For this review, take the finished solid that the model builds, in its own axes (mm). Face numbers are marked on the shaded views. Round coordinates to 2 decimals unless told otherwise and drop trailing zeros. Order: outer loops, then holes, each group sorted by start corner. A loop starts at its lowest first (then second) coordinate and runs counter-clockwise, first axis right, second up. Notation, with made-up numbers: (-10.75, -20) -> (32.25, -20) arc R22 cw to (32.25, 15) -> close; hole circle Ø4 at (6, 67.5). An arc over 180 degrees is marked (long way). Use a Markdown table: item, result. Add a question column.
1) Clearance check with flat-ended pins moving along their axes: P1, Ø2, axis at x = -232, z = -14.5, coming from the +Y side; P2, Ø1, axis at x = -254, z = -40, coming from the -Y side; P3, Ø12, axis at x = -193.5, y = 17, coming from the +Z side (3 decimals). State where each tip first meets the part, or that it passes through.
2) Wall thickness on line 1 along X through (y, z) = (-27, 65); line 2 along Y through (x, z) = (-233.5, 6.5); line 3 along Z through (x, y) = (-229.5, 36): over which ranges is each line inside the solid? List them lowest first. Write a range as [from, to].
3) Consider section D-D (x = -282.5). State the section outline as (y, z) points, plus the area to 3 significant figures.
4) Draft analysis for pull direction X (two halves, no side actions). For the marked faces 1, 2 and 3, state which applies: pulls with the +X half, pulls with the -X half, needs draft (parallel to the pull), parting line crosses it, or undercut.
5) Consider section A-A (z = 59.5). State the section outline as (x, y) points.
6) Consider section B-B (y = 0). State the section outline as (x, z) points.
7) Consider section C-C (z = 25). State the section outline as (x, y) points, plus the area to 3 significant figures.
```python
from build123d import *

# Parameters (mm, degrees)
SKETCH_1_4_R        = 75
BOSS_EXTRUDE1_DEPTH = 18
SKETCH_1_3_R        = 50
BOSS_EXTRUDE2_DEPTH = 311
BOSS_EXTRUDE3_START = -329
SKETCH_1_4_2_R      = 75
BOSS_EXTRUDE3_DEPTH = 18


with BuildPart() as part:
    # Sketch 1_4 → Boss-Extrude1 (new body)
    with BuildSketch(Plane(origin=(0, 0, 0), x_dir=(0, 0, -1), z_dir=(1, 0, 0))):
        Circle(SKETCH_1_4_R)
    extrude(amount=BOSS_EXTRUDE1_DEPTH)

    # 草图1<3> → Boss-Extrude2 (add)
    with BuildSketch(Plane(origin=(0, 0, 0), x_dir=(0, 0, -1), z_dir=(1, 0, 0))):
        Circle(SKETCH_1_3_R)
    extrude(amount=-BOSS_EXTRUDE2_DEPTH)

    # Sketch 1_4 2 → Boss-Extrude3 (add)
    with BuildSketch(Plane(origin=(0, 0, 0), x_dir=(0, 0, -1), z_dir=(1, 0, 0)).offset(BOSS_EXTRUDE3_START)):
        Circle(SKETCH_1_4_2_R)
    extrude(amount=BOSS_EXTRUDE3_DEPTH)


solid = part.part
```
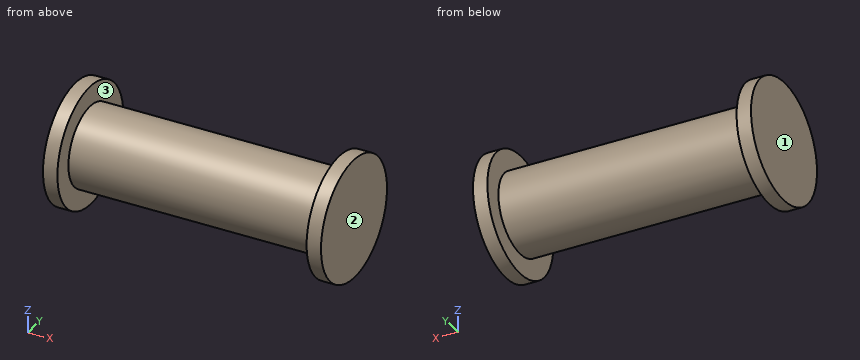
Results list:
| question | item | result |
|---|---|---|
| 1 | P1 | y = 48.14 |
| 1 | P2 | y = -30.66 |
| 1 | P3 | z = 48.775 |
| 2 | line 1 | [-329, -311], [0, 18] |
| 2 | line 2 | [-49.58, 49.58] |
| 2 | line 3 | [-34.7, 34.7] |
| 3 | outline | circle Ø100 at (0, 0) |
| 3 | area | 7,850 mm2 |
| 4 | face 1 | pulls with the -X half |
| 4 | face 2 | pulls with the +X half |
| 4 | face 3 | undercut |
| 5 | outline | (-329, -45.66) -> (-311, -45.66) -> (-311, 45.66) -> (-329, 45.66) -> close; (0, -45.66) -> (18, -45.66) -> (18, 45.66) -> (0, 45.66) -> close |
| 6 | outline | (-329, -75) -> (-311, -75) -> (-311, -50) -> (0, -50) -> (0, -75) -> (18, -75) -> (18, 75) -> (0, 75) -> (0, 50) -> (-311, 50) -> (-311, 75) -> (-329, 75) -> close |
| 7 | outline | (-329, -70.71) -> (-311, -70.71) -> (-311, -43.3) -> (0, -43.3) -> (0, -70.71) -> (18, -70.71) -> (18, 70.71) -> (0, 70.71) -> (0, 43.3) -> (-311, 43.3) -> (-311, 70.71) -> (-329, 70.71) -> close |
| 7 | area | 32,000 mm2 |
